Check sheet for the modelled part. Datum: model origin and axes. Units: mm. Give positions to 0.01 mm unless a question says otherwise; leave off trailing zeros. Order: outer loops, then holes, each group sorted by start corner. A loop starts at its lowest first (then second) coordinate and runs counter-clockwise, first axis right, second up. Notation, with made-up numbers: (78.5, 16) -> (125.5, 16) arc R22 cw to (125.5, 53) -> close; hole circle Ø5 at (2.5, 26.25). An arc over 180 degrees is marked (long way). One line per question, with ' | ' between items.
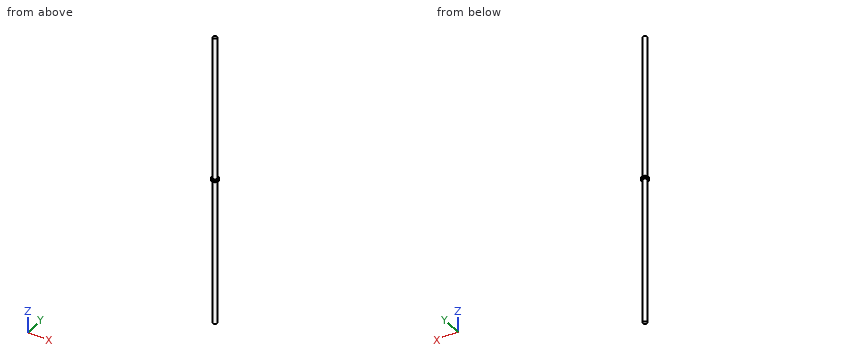
```python
from build123d import *

# Parameters (mm, degrees)
SKETCH_1_W      = 3
SKETCH_1_H      = 430
EXTRUDE_START   = -215
SKETCH_3_R      = 5
EXTRUDE_1_DEPTH = 3


with BuildPart() as part:
    # 草图1 → 旋转1 (revolve)
    with BuildSketch(Plane(origin=(0, 0, 0), x_dir=(1, 0, 0), z_dir=(0, 1, 0))):
        with Locations((1.5, 215)):
            Rectangle(SKETCH_1_W, SKETCH_1_H)
    revolve(axis=Axis((0, 0, 0), (0, 0, -1)))

    # 草图3 → 凸台-拉伸1 (add)
    with BuildSketch(Plane.XY.offset(EXTRUDE_START)):
        Circle(SKETCH_3_R)
    extrude(amount=EXTRUDE_1_DEPTH)


solid = part.part
```
Q1. Section check A-A (x = 0). Enter the section's corners in (y, z).
Result sheet:
outline: (-5, -215) -> (-3, -215) -> (-3, -430) -> (3, -430) -> (3, -215) -> (5, -215) -> (5, -212) -> (3, -212) -> (3, 0) -> (-3, 0) -> (-3, -212) -> (-5, -212) -> close
Q2. Depth check by flat-ended pin: pin 1 Ø6 at (x, z) = (-2, -217) entering from +Y; pin 2 Ø2 at (y, z) = (2, -173.5) entering from -X; pin 3 Ø5 at (x, z) = (1.5, -323.5) entering from -Y; pin 4 Ø6 at (y, z) = (1.5, -347.5) entering from +X. Enter the tip coordinate at first touch or a pass-through.
Result sheet:
pin 1: stops at y = 5 | pin 2: stops at x = -2.83 | pin 3: stops at y = -3 | pin 4: stops at x = 3
Q3. Thickness scan on line 1 (X direction, y = 0.5, z = -112); line 2 (Z direction, x = -0.75, y = 3.5); line 3 (X direction, y = -1, z = -143.5). Record the ranges inside material, lowest first.
Result sheet:
line 1: x = -2.96 to 2.96 | line 2: z = -215 to -212 | line 3: x = -2.83 to 2.83
Q4. Section check C-C (z = -286). Enter the section's corners in (x, y), and give its area (3 significant figures).
Result sheet:
outline: circle Ø6 at (0, 0) | area: 28.3 mm2
